```python
from build123d import *

# Parameters (mm, degrees)
CHAMFER1_SIZE     = 1
HOLE1_D           = 10
HOLE1_DEPTH       = 18
CIRPATTERN1_COUNT = 3


with BuildPart() as part:
    # Sketch2 → Revolve1 (revolve)
    with BuildSketch(Plane.XY, mode=Mode.PRIVATE) as revolve1_sk:
        Polygon((-18, 90), (-18, 110), (18, 110), (18, 90), (11, 90), (11, 93), (-11, 93), (-11, 90), align=None)
    revolve(revolve1_sk.sketch.rotate(Axis((-24.332542805, 0, 0), (1, 0, 0)), 90), axis=Axis((-24.332542805, 0, 0), (1, 0, 0)))

    # Chamfer1
    chamfer1_edges = [part.edges().sort_by_distance(p)[0] for p in [
        (-18, 0, -110),
        (-18, 0, -90),
        (18, 0, -90),
        (18, 0, -110),
    ]]
    chamfer(chamfer1_edges, length=CHAMFER1_SIZE)

    # Hole1
    with Locations(Plane.XY.offset(110)):
        with Locations((0, 0)):
            hole1 = Hole(HOLE1_D / 2, depth=HOLE1_DEPTH)

    # CirPattern1: Hole1 ×3 about axis
    cirpattern1_axis = Axis((17, 0, 0), (-1, 0, 0))
    for i in range(1, CIRPATTERN1_COUNT):
        add(hole1.rotate(cirpattern1_axis, i * 360 / CIRPATTERN1_COUNT), mode=Mode.SUBTRACT)


solid = part.part
```
Geometry check sheet. Reference: the model listing, model coordinates, mm. A direction names the side the tool comes from. Round coordinates to 2 decimals unless told otherwise and drop trailing zeros. Loops run counter-clockwise (first coordinate to the right, second up) from the corner with the lowest first, then second, coordinate; pieces in that order, holes last. Notation, with made-up numbers: (45, -22.75) -> (75, -22.75) arc R23 ccw to (75, 13.25) -> close; hole circle Ø9 at (35, 2). An arc over 180 degrees is marked (long way). Use a Markdown table: item, result.
(1) Sectioned sample at B-B (x = 0.5). Enter the section's corners in (y, z) (3 decimals).
Calculated:
| item | result |
|---|---|
| outline | (-97.653, -50.635) -> (-82.913, -42.125) arc R93 cw to (-4.975, 92.867) -> (-4.975, 109.887) arc R110 ccw to start; (-92.678, -59.252) arc R110 ccw to (92.678, -59.252) -> (77.938, -50.742) arc R93 cw to (-77.938, -50.742) -> close; (4.975, 92.867) arc R93 cw to (82.913, -42.125) -> (97.653, -50.635) arc R110 ccw to (4.975, 109.887) -> close |
(2) Set-up check for faces 1 (the flat face through (11, -76, 49)), 2 (the flat face through (18, 88, -25)), 3 (the cylindrical face through (-4.77, 1.5, 101.31)): record each of +Z, -Z, +X, -X, +Y, -Y from which the full face is reachable in a straight line by a thin tool's end or side.
Calculated:
| item | result |
|---|---|
| face 1 | none |
| face 2 | +Z, -Z, +X, +Y, -Y |
| face 3 | +Z |
(3) Mould release check, pull along Z, two halves, no side actions. Record for faces 4 (the cylindrical face through (-2.307, -85.522, -54.498)), 5 (the flat face through (-18, 88, 25)), 6 (the cylindrical face through (1.08, 90.18, -46.43)), 7 (the cylindrical face through (0.24, 97.59, 50.76)): released by +Z, released by -Z, zero draft, split by the parting line, or undercut.
Calculated:
| item | result |
|---|---|
| face 4 | undercut |
| face 5 | zero draft |
| face 6 | undercut |
| face 7 | split by the parting line |
(4) Go/stop test with flat-tipped pins: P1, Ø8, axis at x = 0, y = 0, coming from the +Z side; P2, Ø1.5, axis at x = 2.5, z = 61, coming from the -Y side; P3, Ø8, axis at x = 0, z = 22.5, coming from the -Y side. Record where each tip stops, or that it passes through.
Calculated:
| item | result |
|---|---|
| P1 | z = -92.91 |
| P2 | y = -92.03 |
| P3 | y = -108.43 |
(5) Sectioned sample at C-C (z = 0). Enter the section's corners in (x, y), then the cut area to 3 significant figures.
Calculated:
| item | result |
|---|---|
| outline | (-18, -109) -> (-17, -110) -> (17, -110) -> (18, -109) -> (18, -91) -> (17, -90) -> (11, -90) -> (11, -93) -> (-11, -93) -> (-11, -90) -> (-17, -90) -> (-18, -91) -> close; (-18, 91) -> (-17, 90) -> (-11, 90) -> (-11, 93) -> (11, 93) -> (11, 90) -> (17, 90) -> (18, 91) -> (18, 109) -> (17, 110) -> (-17, 110) -> (-18, 109) -> close |
| area | 1,300 mm² |
(6) Sectioned sample at A-A (y = 0). Enter the section's corners in (x, z).
Calculated:
| item | result |
|---|---|
| outline | (-18, -109) -> (-17, -110) -> (17, -110) -> (18, -109) -> (18, -91) -> (17, -90) -> (11, -90) -> (11, -93) -> (-11, -93) -> (-11, -90) -> (-17, -90) -> (-18, -91) -> close; (-18, 91) -> (-17, 90) -> (-11, 90) -> (-11, 93) -> (-5, 93) -> (-5, 110) -> (-17, 110) -> (-18, 109) -> close; (5, 93) -> (11, 93) -> (11, 90) -> (17, 90) -> (18, 91) -> (18, 109) -> (17, 110) -> (5, 110) -> close |
(7) Scan lines: probe 1 along Z at (x, y) = (-8, 39.5); probe 2 along Y at (x, z) = (0, 100); probe 3 along Y at (x, z) = (-11.5, 17). Record each from-to range of solid material in increasing order.
Calculated:
| item | result |
|---|---|
| probe 1 | -102.66 to -84.19, 84.19 to 102.66 |
| probe 2 | -45.83 to -5, 5 to 45.83 |
| probe 3 | -108.68 to -88.38, 88.38 to 108.68 |
